Read the model definition and answer for the solid it produces. Units are mm, in the model's axes. A direction names the side the tool comes from. Round coordinates to 2 decimals unless told otherwise and drop trailing zeros. Order: outer loops, then holes, each group sorted by start corner. A loop starts at its lowest first (then second) coordinate and runs counter-clockwise, first axis right, second up.
from build123d import *

# Parameters (mm, degrees)
SKETCH_2_W          = 120
SKETCH_2_H          = 50
EXTRUDE_1_DEPTH     = 50
SKETCH_3_R          = 37.5
CUT_EXTRUDE_1_DEPTH = 139
FILLET_1_R          = 10
SKETCH_4_W          = 30
SKETCH_4_H          = 50
EXTRUDE_2_DEPTH     = 20
EXTRUDE_START       = 3
EXTRUDE_3_DEPTH     = 3
SKETCH_6_R          = 5
CUT_EXTRUDE_2_DEPTH = 38


with BuildPart() as part:
    # 草图2 → 凸台-拉伸1 (new body)
    with BuildSketch(Plane(origin=(0, 0, 0), x_dir=(1, 0, 0), z_dir=(0, 1, 0))):
        Rectangle(SKETCH_2_W, SKETCH_2_H)
    extrude(amount=EXTRUDE_1_DEPTH)

    # 草图3 → 切除-拉伸1 (cut)
    with BuildSketch(Plane.XY.offset(25)):
        Circle(SKETCH_3_R)
    extrude(amount=-CUT_EXTRUDE_1_DEPTH, mode=Mode.SUBTRACT)

    # 圆角1
    fillet_1_edges = [part.edges().sort_by_distance(p)[0] for p in [
        (60, 50, 0),
        (-60, 50, 0),
    ]]
    fillet(fillet_1_edges, radius=FILLET_1_R)

    # 草图4 → 凸台-拉伸2 (add)
    with BuildSketch(Plane.XZ):
        with Locations((-75, 0)):
            Rectangle(SKETCH_4_W, SKETCH_4_H)
        with Locations((75, 0)):
            Rectangle(SKETCH_4_W, SKETCH_4_H)
    extrude(amount=-EXTRUDE_2_DEPTH)

    # 草图5 → 凸台-拉伸3 (add)
    with BuildSketch(Plane.XY.offset(25).offset(EXTRUDE_START)):
        with BuildLine():
            Line((-45, 0), (-37.5, 0))
            ThreePointArc((-37.5, 0), (0, 37.5), (37.5, 0))
            Line((37.5, 0), (45, 0))
            ThreePointArc((45, 0), (0, 45), (-45, 0))
        make_face()
    extrude_3 = extrude(amount=-EXTRUDE_3_DEPTH)

    # 镜向1: 凸台-拉伸3 across plane
    add(extrude_3.mirror(Plane.XY))

    # 草图6 → 切除-拉伸2 (cut)
    with BuildSketch(Plane(origin=(0, 20, 0), x_dir=(1, 0, 0), z_dir=(0, 1, 0))):
        with Locations(Location((-75, 12.5, 0), (0, 0, 270))):
            Circle(SKETCH_6_R)
        with Locations(Location((-75, -12.5, 0), (0, 0, 270))):
            Circle(SKETCH_6_R)
        with Locations(Location((75, -12.5, 0), (0, 0, 90))):
            Circle(SKETCH_6_R)
        with Locations(Location((75, 12.5, 0), (0, 0, 90))):
            Circle(SKETCH_6_R)
    extrude(amount=-CUT_EXTRUDE_2_DEPTH, mode=Mode.SUBTRACT)


solid = part.part
Q1. A cutting plane is placed at C-C, the plane x = 75. Give the vertices of the cut face in (y, z).
Outcome:
outline: (0, -25) - (20, -25) - (20, -17.5) - (0, -17.5) - close; (0, -7.5) - (20, -7.5) - (20, 7.5) - (0, 7.5) - close; (0, 17.5) - (20, 17.5) - (20, 25) - (0, 25) - close
Q2. A cutting plane is placed at D-D, the plane z = 4.5. Give the vertices of the cut face in (x, y).
Outcome:
outline: (-90, 0) - (-37.5, 0) arc R37.5 cw to (37.5, 0) - (90, 0) - (90, 20) - (60, 20) - (60, 40) arc R10 ccw to (50, 50) - (-50, 50) arc R10 ccw to (-60, 40) - (-60, 20) - (-90, 20) - close
Q3. Straight lines are drawn through the part: probe 1 along Z at (x, y) = (75, 13); probe 2 along X at (y, z) = (18, -15); probe 3 along X at (y, z) = (15.25, -12.5). For each, find the intervals that lie inside material, in ascending order.
Outcome:
probe 1: z = -25 to -17.5, -7.5 to 7.5, 17.5 to 25
probe 2: x = -90 to -79.33, -70.67 to -32.9, 32.9 to 70.67, 79.33 to 90
probe 3: x = -90 to -80, -70 to -34.26, 34.26 to 70, 80 to 90
Q4. For a pull along X with two mould halves and no side action, classify faces 4 (the face through (79.88, 10.14, -11.42)), 5 (the face through (-4, 38, -28)), 6 (the face through (56.99, 47.15, -0.35)) as released by +X, released by -X, zero draft, split by the parting line, or undercut.
Outcome:
face 4: undercut
face 5: zero draft
face 6: released by +X
Q5. A cutting plane is placed at A-A, the plane z = -12.5. Give the vertices of the cut face in (x, y).
Outcome:
outline: (-90, 0) - (-80, 0) - (-80, 20) - (-90, 20) - close; (-70, 0) - (-37.5, 0) arc R37.5 cw to (37.5, 0) - (70, 0) - (70, 20) - (60, 20) - (60, 40) arc R10 ccw to (50, 50) - (-50, 50) arc R10 ccw to (-60, 40) - (-60, 20) - (-70, 20) - close; (80, 0) - (90, 0) - (90, 20) - (80, 20) - close
Q6. A cutting plane is placed at B-B, the plane y = 9.5. Give the vertices of the cut face in (x, z), plus the area to 3 significant figures.
Outcome:
outline: (-90, -25) - (-43.99, -25) - (-43.99, -28) - (-36.28, -28) - (-36.28, 28) - (-43.99, 28) - (-43.99, 25) - (-90, 25) - close; (36.28, -28) - (43.99, -28) - (43.99, -25) - (90, -25) - (90, 25) - (43.99, 25) - (43.99, 28) - (36.28, 28) - close; hole circle Ø10 at (-75, -12.5); hole circle Ø10 at (-75, 12.5); hole circle Ø10 at (75, -12.5); hole circle Ø10 at (75, 12.5)
area: 5,150 mm2
Q7. For faces 1 (the face through (75, 20, 0)), 2 (the face through (0.99, 44.99, 26.52)), 3 (the face through (-75, 20, 0)), determine the directions among +Z, -Z, +X, -X, +Y, -Y from which every point of the face is accessible in a straight line to the end or side of a thin tool.
Outcome:
face 1: +Z, -Z, +X, +Y
face 2: +Z, +Y
face 3: +Z, -Z, -X, +Y
Q8. Flat-ended cylindrical pins translate along their axes: pin 1 (24 mm diameter, centred on x = -69.5, z = -11, fed in from +Y); pin 2 (10 mm diameter, centred on y = 39.5, z = -2.5, fed in from -X); pin 3 (15 mm diameter, centred on x = 77, z = -5.5, fed in from +Y). Find the tip coordinate at first contact, or state that the pin passes through.
Outcome:
pin 1: stops at y = 46.61
pin 2: stops at x = -60
pin 3: stops at y = 20
